Design review of the part shown in the three views and the two pictorial views. Dimensions are in mm from the part's minimum x, y and z. Give positions to 0.01 mm unless a question says otherwise; leave off trailing zeros. Order: outer loops, then holes, each group sorted by start corner. A loop starts at its lowest first (then second) coordinate and runs counter-clockwise, first axis right, second up.
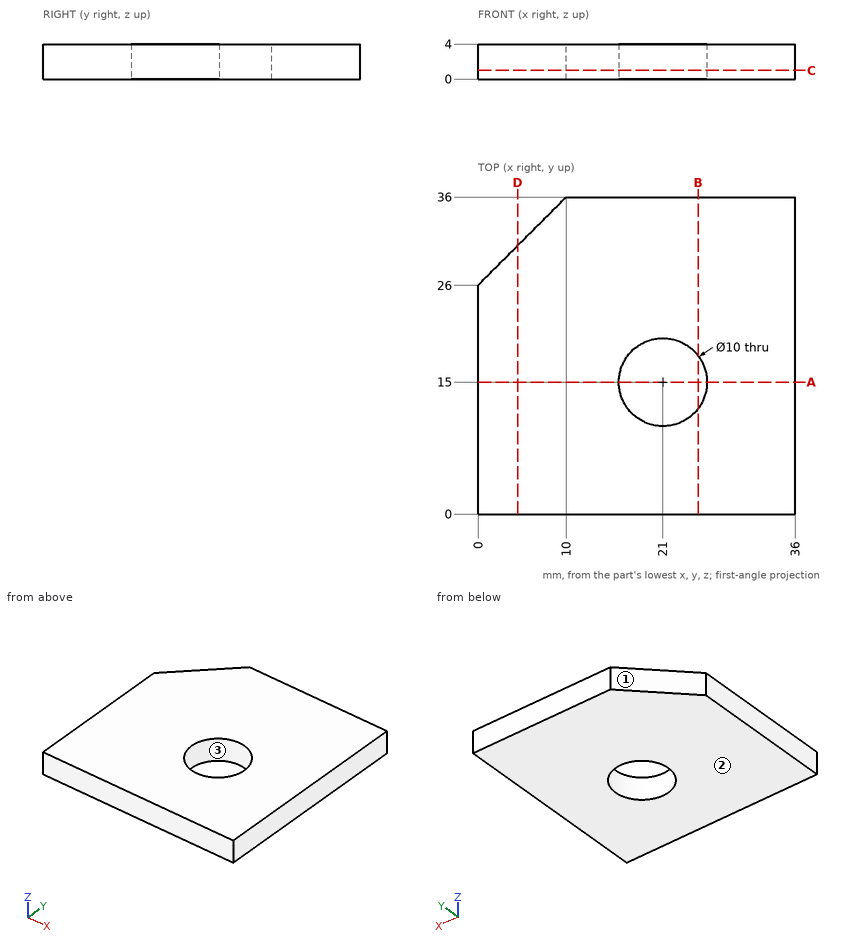
1) We need section C-C on z = 1. Give the boundary of the cut face in (x, y).
Answer sheet:
outline: (0, 0) - (36, 0) - (36, 36) - (10, 36) - (0, 26) - close; hole circle Ø10 at (21, 15)
2) We need section D-D on x = 4.5. Give the boundary of the cut face in (y, z).
Answer sheet:
outline: (0, 0) - (30.5, 0) - (30.5, 4) - (0, 4) - close
3) We need section B-B on x = 25. Give the boundary of the cut face in (y, z), then the cut area to 3 significant figures.
Answer sheet:
outline: (0, 0) - (12, 0) - (12, 4) - (0, 4) - close; (18, 0) - (36, 0) - (36, 4) - (18, 4) - close
area: 120 mm2
4) We need section A-A on y = 15. Give the boundary of the cut face in (x, z), then the cut area to 3 significant figures.
Answer sheet:
outline: (0, 0) - (16, 0) - (16, 4) - (0, 4) - close; (26, 0) - (36, 0) - (36, 4) - (26, 4) - close
area: 104 mm2
5) To check wall thickness, follow line 1 (Y direction, x = 21, z = 2.4); line 2 (X direction, y = 11.5, z = 1.15); line 3 (Y direction, x = 22, z = 1.75). State the ranges of each line that lie inside material, in increasing order.
Answer sheet:
line 1: y = 0 to 10, 20 to 36
line 2: x = 0 to 17.43, 24.57 to 36
line 3: y = 0 to 10.1, 19.9 to 36
6) Draft analysis for pull direction X (two halves, no side actions). For the marked faces 1, 2 and 3, state which applies: +X half, -X half, draft (parallel to the pull), parting line (faces both ways), or undercut.
Answer sheet:
face 1: -X half
face 2: draft
face 3: undercut
